from build123d import *

# Parameters (mm, degrees)
BOSS_EXTRUDE1_DEPTH    = 100
M12_TAPPED_HOLE1_D     = 10.2
M12_TAPPED_HOLE1_DEPTH = 29.25
M12_TAPPED_HOLE1_TIP   = 3.064389157
SKETCH5_R              = 10
CUT_EXTRUDE1_DEPTH     = 100


with BuildPart() as part:
    # Sketch1 → Boss-Extrude1 (new body)
    with BuildSketch(Plane.XY):
        with BuildLine():
            Line((0, 0), (0, -120))
            Line((0, -120), (80, -120))
            Line((80, -120), (80, -108))
            Line((80, -108), (22, -108))
            ThreePointArc((22, -108), (14.928932188, -105.071067812), (12, -98))
            Line((12, -98), (12, 0))
            Line((12, 0), (0, 0))
        make_face()
    extrude(amount=BOSS_EXTRUDE1_DEPTH)

    # M12 Tapped Hole1
    with Locations(Plane(origin=(12, 0, 0), x_dir=(0, 0, -1), z_dir=(1, 0, 0))):
        with Locations((-87.5, -22.5), (-12.5, -22.5), (-12.5, -77.5), (-87.5, -77.5)):
            Hole(M12_TAPPED_HOLE1_D / 2, depth=M12_TAPPED_HOLE1_DEPTH)
            with Locations((0, 0, -(M12_TAPPED_HOLE1_DEPTH + M12_TAPPED_HOLE1_TIP / 2))):  # 118° drill point
                Cone(0, M12_TAPPED_HOLE1_D / 2, M12_TAPPED_HOLE1_TIP, mode=Mode.SUBTRACT)

    # Sketch5 → Cut-Extrude1 (cut)
    with BuildSketch(Plane(origin=(0, -108, 0), x_dir=(1, 0, 0), z_dir=(0, 1, 0))):
        with Locations(Location((46, -50, 0), (0, 0, 270))):
            Circle(SKETCH5_R)
    extrude(amount=-CUT_EXTRUDE1_DEPTH, mode=Mode.SUBTRACT)


solid = part.part
Can you work these out from the model? Positions are in its coordinate system, mm. A direction names the side the tool comes from. Coordinates: 2 decimals unless noted, no trailing zeros. Loops run counter-clockwise (first coordinate to the right, second up) from the corner with the lowest first, then second, coordinate; pieces in that order, holes last. Notation, with made-up numbers: (66, 44.5) - (93, 44.5) arc R16 cw to (93, 65.5) - close; hole circle Ø3 at (13, 27). An arc over 180 degrees is marked (long way). Put each result on its own line as item: value. Start each with the question number.
Item 1: If I drill on line 1 along Z through (x, y) = (6, -77); line 2 along Y through (x, z) = (7, 87.5); line 3 along X through (y, z) = (-116.5, 50), over which ranges is the centre line in solid material (lowest first)?
Item 2: If we mould it in two halves opening along Y, with no side actions, what happens to faces 1 (the face through (5.9, -74.1, 83.7)), 2 (the face through (10, -82, 100)), 3 (the face through (15.01, -105.15, 49.3))? For each: +Y half, -Y half, draft (parallel to the pull), parting line (faces both ways), or undercut.
Item 3: Suppose I cut it at C-C (x = 43). Please give me the cut outline in (y, z), and give its area (3 significant figures).
Item 4: Suppose I cut it at B-B (z = 87.5). Please give me the cut outline in (x, y), and give its area (3 significant figures).
Item 5: Suppose I cut it at D-D (y = -110.5). Please give me the cut outline in (x, z), and give its area (3 significant figures).
Item 6: Which directions (+Z, -Z, +X, -X, +Y, -Y) give clear straight access to the entire face, cutting with the end or side of a thin tool? Please do faces 4 (the face through (10, -82, 0)), 5 (the face through (58, -108, 49)).
Item 7: Suppose I cut it at A-A (y = -22.5). Please give me the cut outline in (x, z).
Item 8: For pin 1 (5 mm diameter, centred on y = -33, z = 26.5, fed in from -X); pin 2 (10 mm diameter, centred on x = 41, y = -99, fed in from -Z); pin 3 (10 mm diameter, centred on x = 25.5, z = 62.5, fed in from +Y); pin 4 (11.5 mm diameter, centred on y = -22.5, z = 12.5, fed in from +X), each with a flat end and sliding along its axis, tell me the tip position at first contact or that it passes through.
Here are the results:
1. line 1: 0 to 7.42, 17.58 to 82.42, 92.58 to 100
1. line 2: -120 to -82.6, -72.4 to -27.6, -17.4 to 0
1. line 3: 0 to 36, 56 to 80
2. face 1: undercut
2. face 2: draft
2. face 3: +Y half
3. outline: (-120, 0) - (-108, 0) - (-108, 40.46) - (-120, 40.46) - close; (-120, 59.54) - (-108, 59.54) - (-108, 100) - (-120, 100) - close
3. area: 971 mm²
4. outline: (0, -120) - (80, -120) - (80, -108) - (22, -108) arc R10 cw to (12, -98) - (12, -82.6) - (0, -82.6) - close; (0, -72.4) - (12, -72.4) - (12, -27.6) - (0, -27.6) - close; (0, -17.4) - (12, -17.4) - (12, 0) - (0, 0) - close
4. area: 2,030 mm²
5. outline: (0, 0) - (80, 0) - (80, 100) - (0, 100) - close; hole circle Ø20 at (46, 50)
5. area: 7,690 mm²
6. face 4: -Z, +X, -X, +Y, -Y
6. face 5: +Z, -Z, +X, +Y
7. outline: (0, 0) - (12, 0) - (12, 7.4) - (0, 7.4) - close; (0, 17.6) - (12, 17.6) - (12, 82.4) - (0, 82.4) - close; (0, 92.6) - (12, 92.6) - (12, 100) - (0, 100) - close
8. pin 1: x = 0
8. pin 2: through
8. pin 3: y = -107.89
8. pin 4: x = 12
